from build123d import *

# Parameters (mm, degrees)
SKETCH1_W               = 134
SKETCH1_H               = 91.5
SKETCH1_R               = 1.6
BOSS_EXTRUDE1_DEPTH     = 2
CUT_EXTRUDE2_DEPTH      = 82.982086458
CUT_EXTRUDE2_DEPTH_BACK = 82.982086458
R2_FILLET_1_R           = 2


with BuildPart() as part:
    # Sketch1 → Boss-Extrude1 (new body)
    with BuildSketch(Plane(origin=(0, 0, 0), x_dir=(1, 0, 0), z_dir=(0, 1, 0))):
        with Locations((1, 0)):
            Rectangle(SKETCH1_W, SKETCH1_H)
        with Locations(Location((-59.5, 31, 0), (0, 0, 270))):
            Circle(SKETCH1_R, mode=Mode.SUBTRACT)
        with Locations(Location((-59.5, 18, 0), (0, 0, 270))):
            Circle(SKETCH1_R, mode=Mode.SUBTRACT)
        with Locations(Location((-59.5, -18, 0), (0, 0, 90))):
            Circle(SKETCH1_R, mode=Mode.SUBTRACT)
        with Locations(Location((-59.5, -31, 0), (0, 0, 90))):
            Circle(SKETCH1_R, mode=Mode.SUBTRACT)
        with Locations(Location((63.5, 3.75, 0), (0, 0, 270))):
            Circle(SKETCH1_R, mode=Mode.SUBTRACT)
        with Locations(Location((63.5, -6.25, 0), (0, 0, 270))):
            Circle(SKETCH1_R, mode=Mode.SUBTRACT)
        with Locations(Location((0.5, -41.25, 0), (0, 0, 270))):
            Circle(SKETCH1_R, mode=Mode.SUBTRACT)
        with Locations(Location((10.5, -41.25, 0), (0, 0, 270))):
            Circle(SKETCH1_R, mode=Mode.SUBTRACT)
        with Locations(Location((10.5, 41.25, 0), (0, 0, 90))):
            Circle(SKETCH1_R, mode=Mode.SUBTRACT)
        with Locations(Location((0.5, 41.25, 0), (0, 0, 90))):
            Circle(SKETCH1_R, mode=Mode.SUBTRACT)
    extrude(amount=BOSS_EXTRUDE1_DEPTH)

    # Sketch5 → Cut-Extrude2 (cut, two sides: drawn at the far end of the back side and taken through both)
    with BuildSketch(Plane(origin=(0, 2, 0), x_dir=(1, 0, 0), z_dir=(0, 1, 0)).offset(-CUT_EXTRUDE2_DEPTH_BACK)):
        with BuildLine():
            Line((-49.255641565, 34.099169914), (-46.471955987, 35.999970141))
            ThreePointArc((-46.471955987, 35.999970141), (-40.91297049, 34.952267774), (-41.960672856, 29.393282278))
            Line((-41.960672856, 29.393282278), (-44.744358435, 27.492482051))
            ThreePointArc((-44.744358435, 27.492482051), (-50.303343931, 28.540184417), (-49.255641565, 34.099169914))
        make_face()
        with BuildLine():
            Line((-49.255641565, 15.935756946), (-19.871985084, 35.999970141))
            ThreePointArc((-19.871985084, 35.999970141), (-14.312999587, 34.952267774), (-15.360701954, 29.393282278))
            Line((-15.360701954, 29.393282278), (-44.744358435, 9.329069084))
            ThreePointArc((-44.744358435, 9.329069084), (-50.303343931, 10.37677145), (-49.255641565, 15.935756946))
        make_face()
        with BuildLine():
            Line((-49.255641565, -2.227656021), (6.727985819, 35.999970141))
            ThreePointArc((6.727985819, 35.999970141), (12.286971315, 34.952267774), (11.239268949, 29.393282278))
            Line((11.239268949, 29.393282278), (-44.744358435, -8.834343884))
            ThreePointArc((-44.744358435, -8.834343884), (-50.303343931, -7.786641517), (-49.255641565, -2.227656021))
        make_face()
        with BuildLine():
            Line((-49.255641565, -20.391068988), (33.327956722, 35.999970141))
            ThreePointArc((33.327956722, 35.999970141), (38.886942218, 34.952267774), (37.839239852, 29.393282278))
            Line((37.839239852, 29.393282278), (-44.744358435, -26.997756851))
            ThreePointArc((-44.744358435, -26.997756851), (-50.303343931, -25.950054485), (-49.255641565, -20.391068988))
        make_face()
        with BuildLine():
            Line((-35.955656114, -29.472775472), (46.627942173, 26.918263657))
            ThreePointArc((46.627942173, 26.918263657), (52.18692767, 25.870561291), (51.139225303, 20.311575794))
            Line((51.139225303, 20.311575794), (-31.444372983, -36.079463334))
            ThreePointArc((-31.444372983, -36.079463334), (-37.00335848, -35.031760968), (-35.955656114, -29.472775472))
        make_face()
        with BuildLine():
            Line((-9.355685211, -29.472775472), (46.627942173, 8.75485069))
            ThreePointArc((46.627942173, 8.75485069), (52.18692767, 7.707148324), (51.139225303, 2.148162827))
            Line((51.139225303, 2.148162827), (-4.844402081, -36.079463334))
            ThreePointArc((-4.844402081, -36.079463334), (-10.403387577, -35.031760968), (-9.355685211, -29.472775472))
        make_face()
        with BuildLine():
            Line((17.244285692, -29.472775472), (46.627942173, -9.408562277))
            ThreePointArc((46.627942173, -9.408562277), (52.18692767, -10.456264644), (51.139225303, -16.01525014))
            Line((51.139225303, -16.01525014), (21.755568822, -36.079463334))
            ThreePointArc((21.755568822, -36.079463334), (16.196583325, -35.031760968), (17.244285692, -29.472775472))
        make_face()
        with BuildLine():
            Line((43.844256595, -29.472775472), (46.627942173, -27.571975244))
            ThreePointArc((46.627942173, -27.571975244), (52.18692767, -28.619677611), (51.139225303, -34.178663107))
            Line((51.139225303, -34.178663107), (48.355539725, -36.079463334))
            ThreePointArc((48.355539725, -36.079463334), (42.796554228, -35.031760968), (43.844256595, -29.472775472))
        make_face()
    extrude(amount=CUT_EXTRUDE2_DEPTH + CUT_EXTRUDE2_DEPTH_BACK, mode=Mode.SUBTRACT)

    # R2 Fillet 1
    r2_fillet_1_edges = [part.edges().sort_by_distance(p)[0] for p in [
        (-66, 1, -45.75),
        (68, 1, -45.75),
        (68, 1, 45.75),
        (-66, 1, 45.75),
    ]]
    fillet(r2_fillet_1_edges, radius=R2_FILLET_1_R)


solid = part.part
Geometry check sheet. Reference: the model listing, model coordinates, mm. Round coordinates to 2 decimals unless told otherwise and drop trailing zeros. Order: outer loops, then holes, each group sorted by start corner. A loop starts at its lowest first (then second) coordinate and runs counter-clockwise, first axis right, second up. Notation, with made-up numbers: (11, 48.5) - (45, 48.5) arc R27 ccw to (45, 82.5) - close; hole circle Ø6 at (2, 16.25). An arc over 180 degrees is marked (long way). One line per question, with ' | ' between items. Start each with the question number.
(1) Sectioned sample at B-B on x = 63.5. Record the cut outline in (y, z).
(2) Sectioned sample at D-D on z = 31. Record the cut outline in (x, y).
(3) Sectioned sample at A-A on z = 41.25. Record the cut outline in (x, y).
(4) Sectioned sample at C-C on y = 1. Count the separate pieces of the cut face and the enclosed holes in it, and give its area (3 significant figures).
(5) Release check for a two-part mould opening along X. For faces 1 (the cylindrical face through (-0.58, 0.99, -40.07)), 2 (the flat face through (0, 0, -1)) record: released by +X, released by -X, zero draft, split by the parting line, or undercut.
(6) Depth check by flat-ended pin: pin 1 Ø2.5 at (x, z) = (10.5, 41.25) entering from -Y; pin 2 Ø1 at (x, z) = (13.5, -9.5) entering from -Y. Enter the tip coordinate at first touch or a pass-through.
(7) Thickness scan on L1, parallel to X at y = 0.8, z = 41.25; L2, parallel to X at y = 0.15, z = 10.5; L3, parallel to X at y = 0.65, z = -3.75. Record the ranges inside material, lowest first. Write a range as [from, to].
Conclusion:
1) outline: (0, -45.75) - (2, -45.75) - (2, -5.35) - (0, -5.35) - close; (0, -2.15) - (2, -2.15) - (2, 4.65) - (0, 4.65) - close; (0, 7.85) - (2, 7.85) - (2, 45.75) - (0, 45.75) - close
2) outline: (-66, 0) - (-61.1, 0) - (-61.1, 2) - (-66, 2) - close; (-57.9, 0) - (-37.28, 0) - (-37.28, 2) - (-57.9, 2) - close; (-24.01, 0) - (-10.68, 0) - (-10.68, 2) - (-24.01, 2) - close; (2.59, 0) - (15.92, 0) - (15.92, 2) - (2.59, 2) - close; (29.19, 0) - (42.52, 0) - (42.52, 2) - (29.19, 2) - close; (52.88, 0) - (68, 0) - (68, 2) - (52.88, 2) - close
3) outline: (-66, 0) - (-1.1, 0) - (-1.1, 2) - (-66, 2) - close; (2.1, 0) - (8.9, 0) - (8.9, 2) - (2.1, 2) - close; (12.1, 0) - (68, 0) - (68, 2) - (12.1, 2) - close
4) separate pieces: 1 | enclosed holes: 18 | area: 8,470 mm2
5) face 1: undercut | face 2: zero draft
6) pin 1: passes through | pin 2: stops at y = 0
7) L1: x = [-66, -1.1], [2.1, 8.9], [12.1, 68] | L2: x = [-66, -34.77], [-20.58, -8.17], [6.02, 18.43], [32.62, 45.03], [52.22, 68] | L3: x = [-66, -40.5], [-26.31, -13.9], [0.29, 12.7], [26.89, 39.3], [52.5, 61.9], [65.1, 68]
